The listing builds one solid part. Answer for the finished solid, in the listing's coordinates (mm). Give positions to 0.01 mm unless a question says otherwise; leave off trailing zeros. Order: outer loops, then holes, each group sorted by start corner. A loop starts at its lowest first (then second) coordinate and runs counter-clockwise, first axis right, second up. Notation, with made-up numbers: (22, 44.5) - (65, 44.5) arc R28 cw to (65, 66.5) - close; hole circle Ø6 at (63, 77.5). An arc over 180 degrees is marked (long way). Answer as CSV lines item,"result". Start each with the question number.
1. Section A-A on x = 14.5 is taken. Give the vertices of the cut face in (y, z).
2. Section D-D on z = 0.1 is taken. Give the vertices of the cut face in (x, y), and give its area (3 significant figures).
3. Section B-B on y = -10 is taken. Give the vertices of the cut face in (x, z), and give its area (3 significant figures).
4. Section C-C on x = 9 is taken. Give the vertices of the cut face in (y, z), and give its area (3 significant figures).
5. Consider line 1 along X through (y, z) = (9, 0.6); line 2 along Y through (x, z) = (15, 0.1); line 3 along X through (y, z) = (-8.5, -0.35). Determine where each line is inside the solid, lowest interval first. Write a range as [from, to].
6. A flat-ended cylindrical pin translates along its axis: pin 1 (1.5 mm diameter, centred on x = 9.36, y = -16.07, fed in from +Z). Find the tip coordinate at first contact, or state that the pin passes through.
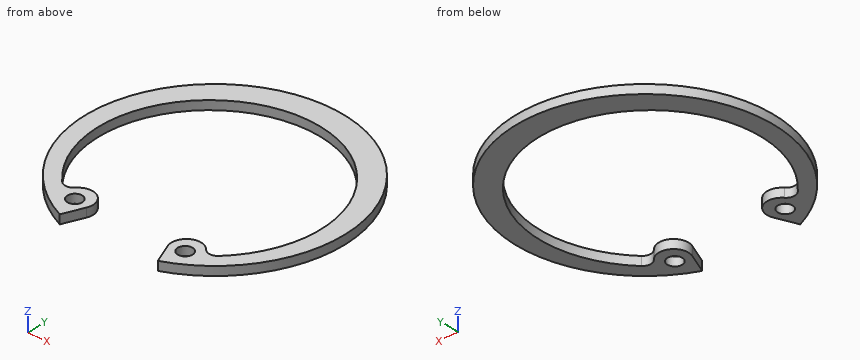
from build123d import *

# Parameters (mm, degrees)
EXTRUDE_962_DEPTH      = 0.75
EXTRUDE_962_DEPTH_BACK = 0.75
SKETCH_1_R             = 1.25


with BuildPart() as part:
    # 草图1 → Extrude 962 (new, two sides: drawn at the far end of the back side and taken through both)
    with BuildSketch(Plane.XY.offset(-EXTRUDE_962_DEPTH_BACK)):
        with BuildLine():
            Line((-6.879499755, -16.608581611), (-8.323364654, -20.094379832))
            ThreePointArc((-8.323364654, -20.094379832), (0, 21.75), (8.323364654, -20.094379832))
            Line((8.323364654, -20.094379832), (6.879499755, -16.608581611))
            ThreePointArc((6.879499755, -16.608581611), (7.876948304, -13.523963446), (11.081029231, -14.017560694))
            ThreePointArc((11.081029231, -14.017560694), (12.16700015, -14.536168573), (13.28459359, -14.08976979))
            ThreePointArc((13.28459359, -14.08976979), (0, 17.65), (-13.28459359, -14.08976979))
            ThreePointArc((-13.28459359, -14.08976979), (-12.16700015, -14.536168573), (-11.081029231, -14.017560694))
            ThreePointArc((-11.081029231, -14.017560694), (-7.876948304, -13.523963446), (-6.879499755, -16.608581611))
        make_face()
        with Locations((-9.363022706, -16.071521577)):
            Circle(SKETCH_1_R, mode=Mode.SUBTRACT)
        with Locations(Location((9.363022706, -16.071521577, 0), (0, 0, 180))):
            Circle(SKETCH_1_R, mode=Mode.SUBTRACT)
    extrude(amount=EXTRUDE_962_DEPTH + EXTRUDE_962_DEPTH_BACK)


solid = part.part
Checks:
1,outline,"(-16.21, -0.75) - (-12.73, -0.75) - (-12.73, 0.75) - (-16.21, 0.75) - close; (10.73, -0.75) - (16.21, -0.75) - (16.21, 0.75) - (10.73, 0.75) - close"
2,outline,"(-13.28, -14.09) arc R18.65 cw (long way) to (13.28, -14.09) arc R1.5 cw to (11.08, -14.02) arc R2.5 ccw to (6.88, -16.61) - (8.32, -20.09) arc R21.75 ccw (long way) to (-8.32, -20.09) - (-6.88, -16.61) arc R2.5 ccw to (-11.08, -14.02) arc R1.5 cw to start; hole circle Ø2.5 at (-9.36, -16.07); hole circle Ø2.5 at (9.36, -16.07)"
2,area,"383 mm²"
3,outline,"(-19.31, -0.75) - (-16.33, -0.75) - (-16.33, 0.75) - (-19.31, 0.75) - close; (16.33, -0.75) - (19.31, -0.75) - (19.31, 0.75) - (16.33, 0.75) - close"
3,area,"8.94 mm²"
4,outline,"(-19.8, -0.75) - (-17.27, -0.75) - (-17.27, 0.75) - (-19.8, 0.75) - close; (-14.88, -0.75) - (-13.16, -0.75) - (-13.16, 0.75) - (-14.88, 0.75) - close; (15.33, -0.75) - (19.8, -0.75) - (19.8, 0.75) - (15.33, 0.75) - close"
4,area,"13.1 mm²"
5,line 1,"x = [-19.8, -15.74], [15.74, 19.8]"
5,line 2,"y = [-15.75, -12.08], [10.08, 15.75]"
5,line 3,"x = [-20.02, -17.08], [17.08, 20.02]"
6,pin 1,"passes through"
